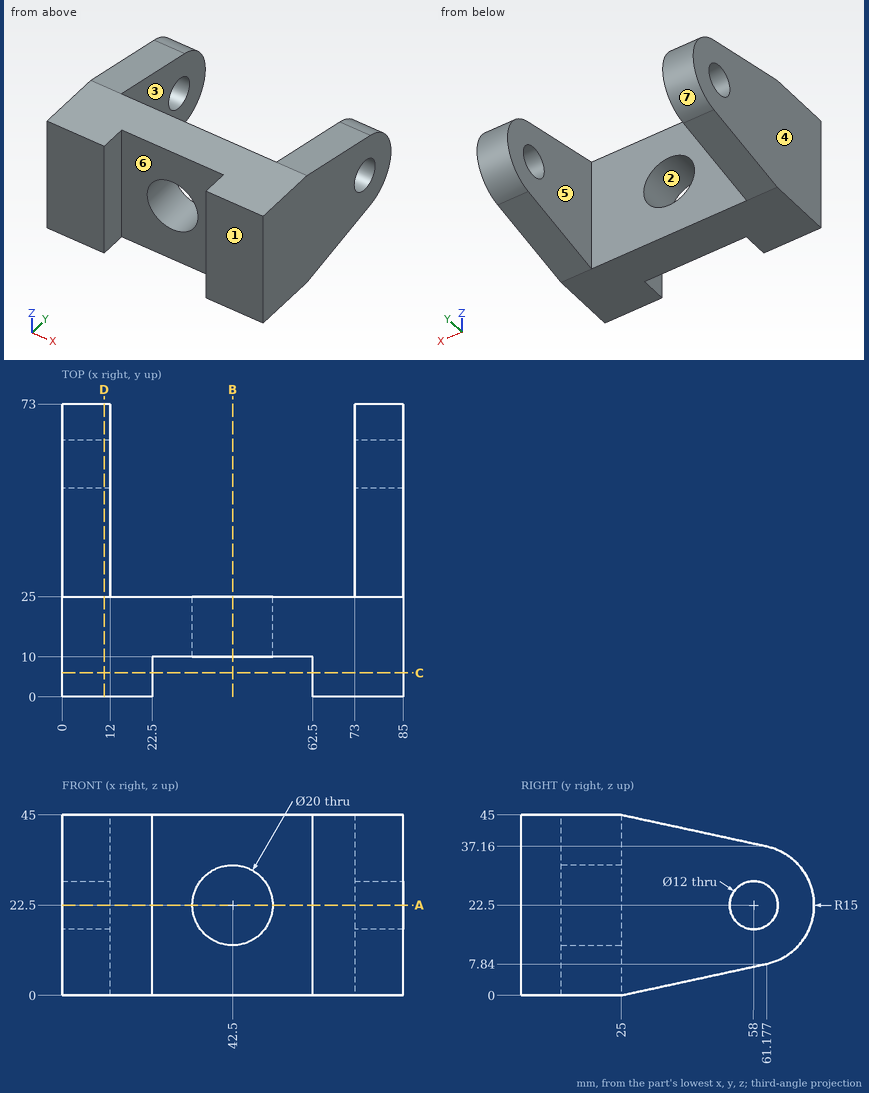
For this review, use the dimensioned drawing (mm, ordinates from the lowest corner) and the shaded views. A direction names the side the tool comes from. Round coordinates to 2 decimals unless told otherwise and drop trailing zeros. Order: outer loops, then holes, each group sorted by start corner. A loop starts at its lowest first (then second) coordinate and runs counter-clockwise, first axis right, second up.
1) Consider section A-A (z = 22.5). State the section outline as (x, y) points.
The answers:
outline: (0, 0) - (22.5, 0) - (22.5, 10) - (32.5, 10) - (32.5, 25) - (12, 25) - (12, 52) - (0, 52) - close; (0, 64) - (12, 64) - (12, 73) - (0, 73) - close; (52.5, 10) - (62.5, 10) - (62.5, 0) - (85, 0) - (85, 52) - (73, 52) - (73, 25) - (52.5, 25) - close; (73, 64) - (85, 64) - (85, 73) - (73, 73) - close
2) For L1, parallel to X at y = 32.5, z = 39.5; L2, parallel to Y at x = 82.75, z = 22.5; L3, parallel to X at y = 15, z = 22, list the stretches that pass through material, from the lowest coordinate up.
The answers:
L1: x = 0 to 12, 73 to 85
L2: y = 0 to 52, 64 to 73
L3: x = 0 to 32.51, 52.49 to 85
3) Draft analysis for pull direction X (two halves, no side actions). For the marked faces 1, 2, 3 and 4, state which applies: released by +X, released by -X, zero draft, split by the parting line, or undercut.
The answers:
face 1: zero draft
face 2: undercut
face 3: undercut
face 4: released by -X
4) Clearance check with a flat-ended pin moving along its axis: pin 1 Ø1.5 at (x, z) = (30.5, 24) entering from +Y. State where the tip first meets the part, or that it passes through.
The answers:
pin 1: stops at y = 25
5) Machinability: for the marked faces 5, 6 and 7, which of the approach directions +Z, -Z, +X, -X, +Y, -Y give a long, thin tool a straight path to every point of the face, cutting with its end or side? Answer none if there is none.
The answers:
face 5: +Z, -Z, +Y
face 6: +Z, -Z, -Y
face 7: +X, -X, +Y
6) Consider section D-D (x = 10.5). State the section outline as (y, z) points.
The answers:
outline: (0, 0) - (25, 0) - (61.18, 7.84) arc R15 ccw to (61.18, 37.16) - (25, 45) - (0, 45) - close; hole circle Ø12 at (58, 22.5)
7) Consider section B-B (x = 42.5). State the section outline as (y, z) points.
The answers:
outline: (10, 0) - (25, 0) - (25, 12.5) - (10, 12.5) - close; (10, 32.5) - (25, 32.5) - (25, 45) - (10, 45) - close
8) Consider section C-C (y = 6). State the section outline as (x, z) points, plus the area to 4 significant figures.
The answers:
outline: (0, 0) - (22.5, 0) - (22.5, 45) - (0, 45) - close; (62.5, 0) - (85, 0) - (85, 45) - (62.5, 45) - close
area: 2,025 mm2
